from build123d import *

# Parameters (mm, degrees)
GB_T_707_1988_HOT_ROLLED_CHANNEL_05_1_DEPTH = 684


with BuildPart() as part:
    # Sketch1 → GB/T 707-1988 hot-rolled channel 05(1) (new body)
    with BuildSketch(Plane.YZ.offset(-342)):
        with BuildLine():
            Line((37, 50), (0, 50))
            Line((0, 50), (0, 0))
            Line((0, 0), (37, 0))
            Line((37, 0), (37, 2.140642022))
            ThreePointArc((37, 2.140642022), (36.101006889, 4.482599144), (33.865849621, 5.621468656))
            Line((33.865849621, 5.621468656), (10.768300757, 8.049118866))
            ThreePointArc((10.768300757, 8.049118866), (6.297986222, 10.326857889), (4.5, 15.010772133))
            Line((4.5, 15.010772133), (4.5, 34.989227867))
            ThreePointArc((4.5, 34.989227867), (6.297986222, 39.673142111), (10.768300757, 41.950881134))
            Line((10.768300757, 41.950881134), (33.865849621, 44.378531344))
            ThreePointArc((33.865849621, 44.378531344), (36.101006889, 45.517400856), (37, 47.859357978))
            Line((37, 47.859357978), (37, 50))
        make_face()
    extrude(amount=GB_T_707_1988_HOT_ROLLED_CHANNEL_05_1_DEPTH)


solid = part.part
Design review of the part built by this model. Coordinates are the model's own, in mm. A direction names the side the tool comes from. Coordinates: 2 decimals unless noted, no trailing zeros. Write each loop counter-clockwise with the first axis right and the second up, starting at its lowest first coordinate (ties: lowest second). Pieces come first, ordered by that corner, then holes. Notation, with made-up numbers: (-11, -4) - (47, -4) arc R24 cw to (47, 10) - close; hole circle Ø9 at (50.25, 69). An arc over 180 degrees is marked (long way). One line per item, written item: value.
1) Add section B-B (x = 37). State the section outline as (y, z) points, plus the area to 3 significant figures.
Answer sheet:
outline: (0, 0) - (37, 0) - (37, 2.14) arc R3.5 ccw to (33.87, 5.62) - (10.77, 8.05) arc R7 cw to (4.5, 15.01) - (4.5, 34.99) arc R7 cw to (10.77, 41.95) - (33.87, 44.38) arc R3.5 ccw to (37, 47.86) - (37, 50) - (0, 50) - close
area: 692 mm2
2) For faces 4 (the face through (-4.79, 22.16, 43.15)), 5 (the face through (-5, 0, 25)), list the 3-axis set-ups (+Z, -Z, +X, -X, +Y, -Y) from which the entire face can be reached by the end or side of a thin tool; tool diameter is ignored.
Answer sheet:
face 4: +X, -X, +Y
face 5: +Z, -Z, +X, -X, -Y
3) Add section C-C (z = 27). State the section outline as (x, y) points.
Answer sheet:
outline: (-342, 0) - (342, 0) - (342, 4.5) - (-342, 4.5) - close
4) Mouldability with a two-part tool opening along Z and no side actions: class faces 1 (the face through (-5, 4.5, 25)), 2 (the face through (-342, 3, 23)), 3 (the face through (-5, 19, 50)) as +Z half, -Z half, draft (parallel to the pull), parting line (faces both ways), or undercut.
Answer sheet:
face 1: undercut
face 2: draft
face 3: +Z half
5) To check wall thickness, follow probe 1 along Y at (x, z) = (-92.5, 25.5); probe 2 along Z at (x, y) = (127, 8.5); probe 3 along Z at (x, y) = (7, 19.5). State the ranges of each line that lie inside material, in increasing order.
Answer sheet:
probe 1: y = 0 to 4.5
probe 2: z = 0 to 8.69, 41.31 to 50
probe 3: z = 0 to 7.13, 42.87 to 50
6) Add section A-A (y = 20). State the section outline as (x, z) points, plus the area to 3 significant figures.
Answer sheet:
outline: (-342, 0) - (342, 0) - (342, 7.08) - (-342, 7.08) - close; (-342, 42.92) - (342, 42.92) - (342, 50) - (-342, 50) - close
area: 9,680 mm2
7) Insertion check: pin 1 (12 mm diameter, centred on x = -240, z = 38.5, fed in from -Y); pin 2 (4 mm diameter, centred on x = -11.5, z = 28, fed in from +Y); pin 3 (22 mm diameter, centred on x = -80, z = 27, fed in from +Y). Each pin has a flat end and moves straight along its axis. Give the tip position at first contact, or say it passes through.
Answer sheet:
pin 1: stops at y = 0
pin 2: stops at y = 4.5
pin 3: stops at y = 5.18
